from build123d import *

# Parameters (mm, degrees)
SKETCH_1_W                = 50
SKETCH_1_H                = 30
EXTRUDE_1_DEPTH           = 15
HOLE_WIZARD_1_D           = 6.6
HOLE_WIZARD_1_CBORE_D     = 11
HOLE_WIZARD_1_CBORE_DEPTH = 6.8
CHAMFER_1_SIZE            = 5
CHAMFER_1_SIZE2           = 8.660254038
CHAMFER_2_SIZE            = 0.3


with BuildPart() as part:
    # 草图1 → 凸台-拉伸1 (new body)
    with BuildSketch(Plane.XY):
        Rectangle(SKETCH_1_W, SKETCH_1_H)
    extrude(amount=EXTRUDE_1_DEPTH)

    # 打孔尺寸根据内六角圆柱头螺钉的类型1 (through all)
    with Locations(Plane(origin=(0, 15, 0), x_dir=(1, 0, 0), z_dir=(0, 1, 0))):
        with Locations((-15, -7.5), (15, -7.5)):
            CounterBoreHole(HOLE_WIZARD_1_D / 2, HOLE_WIZARD_1_CBORE_D / 2, HOLE_WIZARD_1_CBORE_DEPTH)

    # 倒角1
    chamfer_1_edges = [part.edges().sort_by_distance(p)[0] for p in [
        (-25, 0, 15),
    ]]
    chamfer_1_side = [part.faces().sort_by_distance(p)[0] for p in [
        (-25, 0, 7.5),
    ]]
    chamfer(chamfer_1_edges, length=CHAMFER_1_SIZE, length2=CHAMFER_1_SIZE2, reference=chamfer_1_side[0])

    # 倒角2
    chamfer_2_edges = [part.edges().sort_by_distance(p)[0] for p in [
        (4.330127019, -15, 15),
        (-25, -15, 5),
        (-20.669872981, -15, 12.5),
        (-25, 15, 5),
        (-20.669872981, 15, 12.5),
        (25, 0, 15),
        (0, -15, 0),
        (-25, 0, 0),
        (0, 15, 0),
        (25, 0, 0),
        (4.330127019, 15, 15),
        (25, -15, 7.5),
        (25, 15, 7.5),
    ]]
    chamfer(chamfer_2_edges, length=CHAMFER_2_SIZE)


solid = part.part
CAD build for the part. Positions are in the model's coordinates, mm. A direction names the side the tool comes from. Coordinates: 2 decimals unless noted, no trailing zeros. Loops run counter-clockwise (first coordinate to the right, second up) from the corner with the lowest first, then second, coordinate; pieces in that order, holes last. Notation, with made-up numbers: (22, 22.5) -> (55, 22.5) arc R16 cw to (55, 36.5) -> close; hole circle Ø6 at (20.25, -3). An arc over 180 degrees is marked (long way). One line per item, written item: value.
1. Drill centre lines: line 1 (Z direction, x = 15, y = -5); line 2 (Z direction, x = -15, y = 12); line 3 (X direction, y = 13, z = 12.5). Where is each one in solid material? Low to high. Write a range as [from, to].
Answers:
line 1: z = [0, 4.2], [10.8, 15]
line 2: z = [0, 2], [13, 15]
line 3: x = [-20.67, -17.29], [-12.71, 12.71], [17.29, 25]
2. Slice it at B-B on y = -6.5. Write the cut outline in (x, z).
Answers:
outline: (-25, 0.3) -> (-24.7, 0) -> (24.7, 0) -> (25, 0.3) -> (25, 14.7) -> (24.7, 15) -> (-16.34, 15) -> (-25, 10) -> close; hole circle Ø6.6 at (-15, 7.5); hole circle Ø6.6 at (15, 7.5)
3. Slice it at A-A on x = 15. Write the cut outline in (y, z).
Answers:
outline: (-15, 0.3) -> (-14.7, 0) -> (14.7, 0) -> (15, 0.3) -> (15, 2) -> (8.2, 2) -> (8.2, 4.2) -> (-15, 4.2) -> close; (-15, 10.8) -> (8.2, 10.8) -> (8.2, 13) -> (15, 13) -> (15, 14.7) -> (14.7, 15) -> (-14.7, 15) -> (-15, 14.7) -> close
4. Which spindle directions (+Z, -Z, +X, -X, +Y, -Y) get a long thin tool onto all of the face, cutting with end or side? Do faces 4 (the face through (18.3, -3.6, 7.4)), 5 (the face through (-15, 8.2, 11)). Say none if no direction does.
Answers:
face 4: +Y, -Y
face 5: +Y
5. Pull direction Z, two halves, no side cores. Call faces 1 (the face through (-25, 0, 5)), 2 (the face through (-20.654, 14.852, 12.333)), 3 (the face through (20.08, 11.65, 9.61)): pulls with the +Z half, pulls with the -Z half, needs draft (parallel to the pull), parting line crosses it, or undercut.
Answers:
face 1: needs draft
face 2: pulls with the +Z half
face 3: undercut
6. Slice it at C-C on z = 7.5. Write the cut outline in (x, y), and give its area (3 significant figures).
Answers:
outline: (-25, -14.7) -> (-24.7, -15) -> (-18.3, -15) -> (-18.3, 8.2) -> (-20.5, 8.2) -> (-20.5, 15) -> (-24.7, 15) -> (-25, 14.7) -> close; (-11.7, -15) -> (11.7, -15) -> (11.7, 8.2) -> (9.5, 8.2) -> (9.5, 15) -> (-9.5, 15) -> (-9.5, 8.2) -> (-11.7, 8.2) -> close; (18.3, -15) -> (24.7, -15) -> (25, -14.7) -> (25, 14.7) -> (24.7, 15) -> (20.5, 15) -> (20.5, 8.2) -> (18.3, 8.2) -> close
area: 1,040 mm^2
7. Slice it at D-D on z = 2.75. Write the cut outline in (x, y), and give its area (3 significant figures).
Answers:
outline: (-25, -14.7) -> (-24.7, -15) -> (24.7, -15) -> (25, -14.7) -> (25, 14.7) -> (24.7, 15) -> (17.77, 15) -> (17.77, 8.2) -> (12.23, 8.2) -> (12.23, 15) -> (-12.23, 15) -> (-12.23, 8.2) -> (-17.77, 8.2) -> (-17.77, 15) -> (-24.7, 15) -> (-25, 14.7) -> close
area: 1,420 mm^2
8. Flat gauge pin, fed straight in: P1, Ø3.5, axis at x = -14, z = 5.5, coming from the +Y side. Where does the tip first touch, or does it go through?
Answers:
P1: stops at y = 8.2
